```python
from build123d import *

# Parameters (mm, degrees)
BASE_BLOCK_DEPTH      = 40
SIDE_SLOT_DEPTH       = 56.466205928
SIDE_SLOT_DEPTH_BACK  = 56.466205928
SIDE_SLOT_SKETCH_W    = 5
SIDE_SLOT_SKETCH_H    = 22
TOP_STEP_POCKET_DEPTH = 6
ARC_RELIEF_CUT_DEPTH  = 30
THROUGH_HOLE_SKETCH_R = 5
THROUGH_HOLE_DEPTH    = 110


with BuildPart() as part:
    # Base Block Profile Sketch → Base Block (new, symmetric)
    with BuildSketch(Plane(origin=(0, 0, 0), x_dir=(1, 0, 0), z_dir=(0, 1, 0))):
        Polygon((11.5, 20.5), (32.5, 5.795641698), (32.5, -20.5), (-32.5, -20.5), (-32.5, 15.5), (-27.5, 20.5), align=None)
    extrude(amount=BASE_BLOCK_DEPTH, both=True)

    # Side Slot Sketch → Side Slot (cut, two sides: drawn at the far end of the back side and taken through both)
    with BuildSketch(Plane.XY.offset(-SIDE_SLOT_DEPTH_BACK)):
        with Locations((30, 0.707540159)):
            Rectangle(SIDE_SLOT_SKETCH_W, SIDE_SLOT_SKETCH_H)
    extrude(amount=SIDE_SLOT_DEPTH + SIDE_SLOT_DEPTH_BACK, mode=Mode.SUBTRACT)

    # Top Step Pocket Sketch → Top Step Pocket (cut)
    with BuildSketch(Plane(origin=(0, 40, 0), x_dir=(1, 0, 0), z_dir=(0, 1, 0))):
        with BuildLine():
            Line((16.483327146, 17.010636767), (11.5, 20.5))
            Line((11.5, 20.5), (-27.5, 20.5))
            Line((-27.5, 20.5), (-32.5, 15.5))
            Line((-32.5, 15.5), (-32.5, -7.5))
            Line((-32.5, -7.5), (-22.5, -7.5))
            ThreePointArc((-22.5, -7.5), (-0.563327522, 0.866615575), (16.483327146, 17.010636767))
        make_face()
    extrude(amount=-TOP_STEP_POCKET_DEPTH, mode=Mode.SUBTRACT)

    # Arc Relief Sketch → Arc Relief Cut (cut, symmetric)
    with BuildSketch(Plane(origin=(0, 0, 0), x_dir=(1, 0, 0), z_dir=(0, 1, 0))):
        with BuildLine():
            Line((-27.5, 20.5), (-32.5, 15.5))
            Line((-32.5, 15.5), (-32.5, -7.5))
            Line((-32.5, -7.5), (-22.5, -7.5))
            ThreePointArc((-22.5, -7.5), (-0.563327522, 0.866615575), (16.483327146, 17.010636767))
            Line((16.483327146, 17.010636767), (11.5, 20.5))
            Line((11.5, 20.5), (-27.5, 20.5))
        make_face()
    extrude(amount=ARC_RELIEF_CUT_DEPTH, both=True, mode=Mode.SUBTRACT)

    # Through Hole Sketch → Through Hole (cut)
    with BuildSketch(Plane(origin=(0, 34, 0), x_dir=(1, 0, 0), z_dir=(0, 1, 0))):
        with Locations(Location((-20.5, 10.5, 0), (0, 0, 270))):
            Circle(THROUGH_HOLE_SKETCH_R)
    extrude(amount=-THROUGH_HOLE_DEPTH, mode=Mode.SUBTRACT)


solid = part.part
```
The model under review builds one solid part; all positions refer to its coordinate system, in mm. A direction names the side the tool comes from. Coordinates: 2 decimals unless noted, no trailing zeros. Write each loop counter-clockwise with the first axis right and the second up, starting at its lowest first coordinate (ties: lowest second). Pieces come first, ordered by that corner, then holes. Notation, with made-up numbers: (-10, 42) -> (27, 42) arc R22 ccw to (27, 70) -> close; hole circle Ø1 at (75, -6.5). An arc over 180 degrees is marked (long way). One line per item, written item: value. Start each with the question number.
Q1. Clearance check with flat-ended pins moving along their axes: P1, Ø1.5, axis at y = -1, z = -4.5, coming from the -X side; P2, Ø1.5, axis at y = 4, z = -7, coming from the -X side; P3, Ø5, axis at x = -26.5, y = 37, coming from the -Z side; P4, Ø8, axis at x = -20.5, z = -10.5, coming from the +Y side. State where each tip first meets the part, or that it passes through.
Q2. The part is to be moulded in two halves that separate along Y. For faces 4 (the face through (30, -10.292, 5)), 5 (the face through (-14, 34, -10)), 6 (the face through (-32.5, -8, 11)), 7 (the face through (-14, 30, -10)), say which applies: +Y half, -Y half, draft (parallel to the pull), parting line (faces both ways), or undercut.
Q3. Add section A-A, the plane z = -10.5. Give the boundary of the cut face in (x, y), then the cut area to 3 significant figures.
Q4. For faces 1 (the face through (-28, 37, 7.5)), 2 (the face through (-28, 0, 7.5)), 3 (the face through (27.5, 1, 5)), list the 3-axis set-ups (+Z, -Z, +X, -X, +Y, -Y) from which the entire face can be reached by the end or side of a thin tool; tool diameter is ignored.
Q5. Add section B-B, the plane z = 16. Give the boundary of the cut face in (x, y), then the cut area to 3 significant figures.
Q6. Add section D-D, the plane y = 1. Give the boundary of the cut face in (x, z), then the cut area to 3 significant figures.
Q7. Add section C-C, the plane x = -20.5. Give the boundary of the cut face in (y, z), then the cut area to 3 significant figures.
Q8. To check wall thickness, follow probe 1 along Y at (x, z) = (12, -13); probe 2 along Y at (x, z) = (28.5, 1.5); probe 3 along X at (y, z) = (5, 16.5). State the ranges of each line that lie inside material, in increasing order.
Response:
1. P1: x = 3.62
1. P2: x = 6.72
1. P3: z = 7.5
1. P4: through
2. face 4: undercut
2. face 5: +Y half
2. face 6: draft
2. face 7: undercut
3. outline: (-32.5, -40) -> (-25.5, -40) -> (-25.5, -30) -> (-32.5, -30) -> close; (-32.5, 30) -> (-25.5, 30) -> (-25.5, 34) -> (-32.5, 34) -> close; (-15.5, -40) -> (25.78, -40) -> (25.78, 40) -> (11.16, 40) -> (11.16, 34) -> (-15.5, 34) -> (-15.5, 30) -> (11.16, 30) -> (11.16, -30) -> (-15.5, -30) -> close
3. area: 1,640 mm²
4. face 1: -Z, -X, +Y
4. face 2: -Z, -X
4. face 3: +Z, -Z, +X
5. outline: (-32.5, -40) -> (32.5, -40) -> (32.5, -10.29) -> (27.5, -10.29) -> (27.5, 11.71) -> (32.5, 11.71) -> (32.5, 40) -> (-32.5, 40) -> close
5. area: 5,090 mm²
6. outline: (-32.5, 7.5) -> (-22.5, 7.5) arc R60 cw to (16.48, -17.01) -> (27.5, -9.3) -> (27.5, 20.5) -> (-32.5, 20.5) -> close
6. area: 1,340 mm²
7. outline: (-40, -20.5) -> (-30, -20.5) -> (-30, -15.5) -> (-40, -15.5) -> close; (-40, -5.5) -> (-30, -5.5) -> (-30, 7.13) -> (30, 7.13) -> (30, -5.5) -> (34, -5.5) -> (34, 7.13) -> (40, 7.13) -> (40, 20.5) -> (-40, 20.5) -> close; (30, -20.5) -> (34, -20.5) -> (34, -15.5) -> (30, -15.5) -> close
7. area: 1,320 mm²
8. probe 1: -40 to -30, 30 to 34
8. probe 2: -40 to -10.29, 11.71 to 40
8. probe 3: -32.5 to 27.5
